from build123d import *

# Parameters (mm, degrees)
HEX_HEAD_50AF_X20_DEPTH = 20
SHANK_SKETCH_20_R       = 10
SHANK_20X80_DEPTH       = 80


with BuildPart() as part:
    # Hex Head Sketch 50AF → Hex Head 50AF x20 (new body)
    with BuildSketch(Plane(origin=(0, 0, 0), x_dir=(1, 0, 0), z_dir=(0, 1, 0))):
        Polygon((28.867513459, 0), (14.43375673, 25), (-14.43375673, 25), (-28.867513459, 0), (-14.43375673, -25), (14.43375673, -25), align=None)
    extrude(amount=HEX_HEAD_50AF_X20_DEPTH)

    # Shank Sketch Ø20 → Shank Ø20x80 (add)
    with BuildSketch(Plane.XZ):
        with Locations(Location((0, 0, 0), (0, 0, 270))):
            Circle(SHANK_SKETCH_20_R)
    extrude(amount=SHANK_20X80_DEPTH)


solid = part.part
Design review of the part built by this model. Coordinates are the model's own, in mm. A direction names the side the tool comes from. Coordinates: 2 decimals unless noted, no trailing zeros. Write each loop counter-clockwise with the first axis right and the second up, starting at its lowest first coordinate (ties: lowest second). Pieces come first, ordered by that corner, then holes. Notation, with made-up numbers: (70, -15.75) -> (78, -15.75) arc R15 cw to (78, 9.25) -> close; hole circle Ø11 at (39, 13). An arc over 180 degrees is marked (long way). Write each question's results on one line, items separated by ' | '. Start each with the question number.
(1) Take a section at D-D on x = -22.5. Write out the cut boundary in (y, z), and give its area (3 significant figures).
(2) Take a section at C-C on y = -17. Write out the cut boundary in (x, z).
(3) Take a section at A-A on x = 0. Write out the cut boundary in (y, z), and give its area (3 significant figures).
(4) Clearance check with flat-ended pins moving along their axes: P1, Ø15, axis at x = 0, z = -11, coming from the -Y side; P2, Ø1, axis at x = -21, y = 8.5, coming from the +Z side; P3, Ø1, axis at x = -7, z = 12.5, coming from the -Y side; P4, Ø10, axis at x = -7.5, y = -69.5, coming from the -Z side. State where each tip first meets the part, or that it passes through.
(5) Take a section at B-B on z = 7. Write out the cut boundary in (x, y).
(6) For line 1 along Y through (x, z) = (-21.5, -9.5); line 2 along X through (y, z) = (12, 19); line 3 along Z through (x, y) = (-5, -59), list the stretches that pass through material, from the lowest coordinate up. Write a range as from..to.
(7) Tool access review of faces 1 (the face through (0, 10, -25)), 2 (the face through (12, 0, 0)): name each direction out of +Z, -Z, +X, -X, +Y, -Y from which nothing blocks a thin tool from reaching the whole face with its end or side.
Results found:
1) outline: (0, -11.03) -> (20, -11.03) -> (20, 11.03) -> (0, 11.03) -> close | area: 441 mm2
2) outline: circle Ø20 at (0, 0)
3) outline: (-80, -10) -> (0, -10) -> (0, -25) -> (20, -25) -> (20, 25) -> (0, 25) -> (0, 10) -> (-80, 10) -> close | area: 2,600 mm2
4) P1: stops at y = -80 | P2: stops at z = 14.49 | P3: stops at y = 0 | P4: stops at z = -9.68
5) outline: (-24.83, 0) -> (-7.14, 0) -> (-7.14, -80) -> (7.14, -80) -> (7.14, 0) -> (24.83, 0) -> (24.83, 20) -> (-24.83, 20) -> close
6) line 1: y = 0..20 | line 2: x = -17.9..17.9 | line 3: z = -8.66..8.66
7) face 1: -Z, +X, -X, +Y, -Y | face 2: -Y
